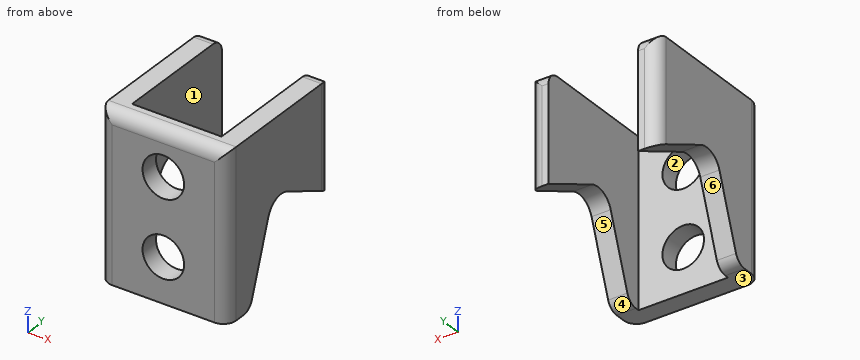
from build123d import *

# Parameters (mm, degrees)
EXTRUDE_1_DEPTH     = 10
SKETCH_2_W          = 26
SKETCH_2_H          = 20
CUT_EXTRUDE_1_DEPTH = 7
CUT_EXTRUDE_2_REACH = 38.125
SKETCH_3_R          = 3.25
FILLET_3_R          = 2


with BuildPart() as part:
    # 草图1 → 凸台-拉伸1 (new, symmetric)
    with BuildSketch(Plane(origin=(0, 0, 0), x_dir=(0, 0, -1), z_dir=(1, 0, 0))):
        with BuildLine():
            Line((17, 23), (0, 23))
            Line((0, 23), (0, 0))
            Line((0, 0), (26, 0))
            Line((26, 0), (26, 5))
            Line((26, 5), (14.014940421, 9.166334948))
            ThreePointArc((14.014940421, 9.166334948), (12.227975796, 10.852881082), (12.300632982, 13.308975821))
            Line((12.300632982, 13.308975821), (17, 23))
        make_face()
    extrude(amount=EXTRUDE_1_DEPTH, both=True)

    # 草图2 → 切除-拉伸1 (cut, symmetric)
    with BuildSketch(Plane(origin=(0, 0, 0), x_dir=(0, 0, -1), z_dir=(1, 0, 0))):
        with Locations((13, 13)):
            Rectangle(SKETCH_2_W, SKETCH_2_H)
    extrude(amount=CUT_EXTRUDE_1_DEPTH, both=True, mode=Mode.SUBTRACT)

    # 草图3 → 切除-拉伸2 (cut, up to next)
    with BuildSketch(Plane.XZ, mode=Mode.PRIVATE) as cut_extrude_2_sk1:
        with Locations(Location((0, -7, 0), (0, 0, 270))):
            Circle(SKETCH_3_R)
    cut_extrude_2_tool1 = extrude(cut_extrude_2_sk1.sketch, amount=-CUT_EXTRUDE_2_REACH, mode=Mode.PRIVATE) & part.part
    # 草图3 → 切除-拉伸2 (cut, up to next)
    with BuildSketch(Plane.XZ, mode=Mode.PRIVATE) as cut_extrude_2_sk2:
        with Locations(Location((0, -19, 0), (0, 0, 270))):
            Circle(SKETCH_3_R)
    cut_extrude_2_tool2 = extrude(cut_extrude_2_sk2.sketch, amount=-CUT_EXTRUDE_2_REACH, mode=Mode.PRIVATE) & part.part
    add(cut_extrude_2_tool1.solids().sort_by_distance((0, 0, -7))[0], mode=Mode.SUBTRACT)
    add(cut_extrude_2_tool2.solids().sort_by_distance((0, 0, -19))[0], mode=Mode.SUBTRACT)

    # 圆角3
    fillet_3_edges = [part.edges().sort_by_distance(p)[0] for p in [
        (-10, 23, -8.5),
        (10, 23, -8.5),
        (8.5, 5, -26),
        (0, 0, 0),
        (8.5, 23, 0),
        (10, 0, -13),
        (-8.5, 5, -26),
        (-8.5, 23, 0),
        (-10, 0, -13),
    ]]
    fillet(fillet_3_edges, radius=FILLET_3_R)


solid = part.part
For this review, take the finished solid that the model builds, in its own axes (mm). Face numbers are marked on the shaded views. A direction names the side the tool comes from. Give positions to 0.01 mm unless a question says otherwise; leave off trailing zeros. Order: outer loops, then holes, each group sorted by start corner. A loop starts at its lowest first (then second) coordinate and runs counter-clockwise, first axis right, second up. Notation, with made-up numbers: M -20,46.5 L -16,46.5 A28 cw -16,67.5 Z; hole C 81.5,28.25 d2. An arc over 180 degrees is marked long. Answer in a Markdown table with one row per item. Add a question column.
(1) Wall thickness on probe 1 along X at (y, z) = (2.1, -7); probe 2 along X at (y, z) = (6, -21.25); probe 3 along Y at (x, z) = (0.5, -3): over which ranges is each line inside the solid? List them lowest first. Write a range as [from, to].
(2) For pin 1 (8.5 mm diameter, centred on x = 0, z = -7, fed in from +Y), flat-tipped, find the tip position at first contact; note if it passes through.
(3) Consider section D-D on x = 6.5. State the section outline as (y, z) points.
(4) Mouldability with a two-part tool opening along Y and no side actions: class the marked faces 3, 4, 5 and 6 as +Y half, -Y half, draft (parallel to the pull), parting line (faces both ways), or undercut.
(5) Consider section B-B on x = 1.25. State the section outline as (y, z) points, and give its area (3 significant figures).
(6) Consider section C-C on y = 19. State the section outline as (x, z) points.
(7) For the marked faces 1 and 2, list the 3-axis set-ups (+Z, -Z, +X, -X, +Y, -Y) from which the entire face can be reached by the end or side of a thin tool; tool diameter is ignored.
(8) Consider section A-A on z = -7. State the section outline as (x, y) points, and give its area (3 significant figures).
Evaluation:
| question | item | result |
|---|---|---|
| 1 | probe 1 | x = [-10, -3.25], [3.25, 10] |
| 1 | probe 2 | x = [-10, -7], [7, 10] |
| 1 | probe 3 | y = [0, 3] |
| 2 | pin 1 | stops at y = 3 |
| 3 | outline | M 0,-26 L 3,-26 L 3,0 L 2,0 A2 ccw 0,-2 Z |
| 4 | face 3 | draft |
| 4 | face 4 | +Y half |
| 4 | face 5 | undercut |
| 4 | face 6 | undercut |
| 5 | outline | M 0,-26 L 3,-26 L 3,-22 L 0,-22 Z; M 0,-16 L 3,-16 L 3,-10 L 0,-10 Z; M 0,-4 L 3,-4 L 3,0 L 2,0 A2 ccw 0,-2 Z |
| 5 | area | 41.1 mm^2 |
| 6 | outline | M -10,-15.06 L -7,-15.06 L -7,0 L -10,0 Z; M 7,-15.06 L 10,-15.06 L 10,0 L 7,0 Z |
| 7 | face 1 | +Z, -Z, +Y |
| 7 | face 2 | +Y, -Y |
| 8 | outline | M -10,2 A2 ccw -8,0 L -3.25,0 L -3.25,3 L -7,3 L -7,23 L -8,23 A2 ccw -10,21 Z; M 3.25,0 L 8,0 A2 ccw 10,2 L 10,21 A2 ccw 8,23 L 7,23 L 7,3 L 3.25,3 Z |
| 8 | area | 157 mm^2 |
